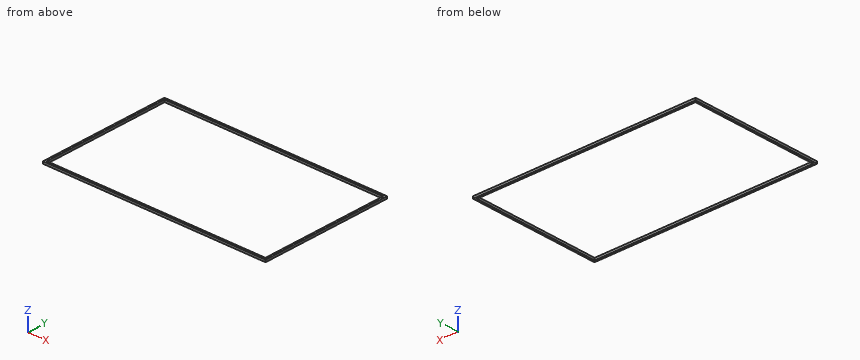
from build123d import *

# Parameters (mm, degrees)
SKETCH_1_W      = 1042
SKETCH_1_H      = 610.2
EXTRUDE_1_DEPTH = 10


with BuildPart() as part:
    # 草图1 → 凸台-拉伸1 (new body)
    with BuildSketch(Plane.XY):
        Polygon((-531, 5), (531, 5), (531, -5), (531, -615.2), (531, -625.2), (-531, -625.2), align=None)
        with Locations((0, -310.1)):
            Rectangle(SKETCH_1_W, SKETCH_1_H, mode=Mode.SUBTRACT)
    extrude(amount=EXTRUDE_1_DEPTH)


solid = part.part
Can you work these out from the model? Positions are in its coordinate system, mm. Coordinates: 2 decimals unless noted, no trailing zeros. Loops run counter-clockwise (first coordinate to the right, second up) from the corner with the lowest first, then second, coordinate; pieces in that order, holes last. Notation, with made-up numbers: (56.5, -40) - (97.5, -40) arc R14 ccw to (97.5, -20) - close; hole circle Ø10 at (60.5, 13.5). An arc over 180 degrees is marked (long way). Answer as a JSON object with one key per item and string values. Group by question number.
Item 1: If I drill on L1, parallel to X at y = -517, z = 3.5; L2, parallel to Y at x = -360, z = 1.25, over which ranges is the centre line in solid material (lowest first)? Write a range as from..to.
Item 2: If we section it at B-B (z = 4.5): List the corners of the cut face in (x, y) for me.
Item 3: If we section it at A-A (y = -271.5): List the corners of the cut face in (x, z) for me.
Item 4: If we section it at C-C (x = -45.5): List the corners of the cut face in (y, z) for me.
Returned:
{
 "1": {"L1": "x = -531..-521, 521..531", "L2": "y = -625.2..-615.2, -5..5"},
 "2": {"outline": "(-531, -625.2) - (531, -625.2) - (531, 5) - (-531, 5) - close; hole (-521, -615.2) - (521, -615.2) - (521, -5) - (-521, -5) - close"},
 "3": {"outline": "(-531, 0) - (-521, 0) - (-521, 10) - (-531, 10) - close; (521, 0) - (531, 0) - (531, 10) - (521, 10) - close"},
 "4": {"outline": "(-625.2, 0) - (-615.2, 0) - (-615.2, 10) - (-625.2, 10) - close; (-5, 0) - (5, 0) - (5, 10) - (-5, 10) - close"}
}
